Design review of the part built by this model. Coordinates are the model's own, in mm. Round coordinates to 2 decimals unless told otherwise and drop trailing zeros. Loops run counter-clockwise (first coordinate to the right, second up) from the corner with the lowest first, then second, coordinate; pieces in that order, holes last. Notation, with made-up numbers: (84, 86.5) -> (121, 86.5) arc R13 cw to (121, 106.5) -> close; hole circle Ø9 at (82, -27). An arc over 180 degrees is marked (long way). Write each question's results on one line, items separated by ' | '. Start each with the question number.
from build123d import *

# Parameters (mm, degrees)
SKETCH1_W                  = 187
SKETCH1_H                  = 137
BOSS_EXTRUDE1_DEPTH        = 4.87
F_7_0_7_DIAMETER_HOLE1_D   = 7
F_3_2_3_2_DIAMETER_HOLE1_D = 3.2
SKETCH6_W                  = 58
SKETCH6_H                  = 101.3
BOSS_EXTRUDE2_DEPTH        = 1
SKETCH7_W                  = 12.3
SKETCH7_H                  = 11
BOSS_EXTRUDE3_DEPTH        = 1
SKETCH8_W                  = 203.41830683
SKETCH8_H                  = 2.7
CUT_EXTRUDE1_DEPTH         = 1
FILLET1_R                  = 7


with BuildPart() as part:
    # Sketch1 → Boss-Extrude1 (new body)
    with BuildSketch(Plane.XY):
        Rectangle(SKETCH1_W, SKETCH1_H)
    extrude(amount=BOSS_EXTRUDE1_DEPTH)

    # Ø7.0 (7) Diameter Hole1 (through all)
    with Locations(Plane.XY.offset(4.87)):
        with Locations((-28.5, 62), (-85.5, 62), (28.5, 62), (85.5, 62), (85.5, -62), (28.5, -62), (-85.5, -62), (-28.5, -62)):
            Hole(F_7_0_7_DIAMETER_HOLE1_D / 2)

    # Ø3.2 (3.2) Diameter Hole1 (through all)
    with Locations(Plane.XY.offset(4.87)):
        with Locations((-57.1, 61.02), (57.1, 60.975), (57.1, -60.975), (-57.1, -61.02)):
            Hole(F_3_2_3_2_DIAMETER_HOLE1_D / 2)

    # Sketch6 → Boss-Extrude2 (add)
    with BuildSketch(Plane.XY.offset(4.87)):
        with Locations((-61, 0)):
            Rectangle(SKETCH6_W, SKETCH6_H)
        Rectangle(SKETCH6_W, SKETCH6_H)
        with Locations((61, 0)):
            Rectangle(SKETCH6_W, SKETCH6_H)
    extrude(amount=BOSS_EXTRUDE2_DEPTH)

    # Sketch7 → Boss-Extrude3 (add)
    with BuildSketch(Plane.XY.offset(4.87)):
        with Locations((-68.55, -57.85)):
            Rectangle(SKETCH7_W, SKETCH7_H)
        with Locations((-45.24, -57.85)):
            Rectangle(SKETCH7_W, SKETCH7_H)
        with Locations((-11.54, -57.85)):
            Rectangle(SKETCH7_W, SKETCH7_H)
    extrude(amount=BOSS_EXTRUDE3_DEPTH)

    # Sketch8 → Cut-Extrude1 (cut)
    with BuildSketch(Plane.XY.offset(5.87)):
        Rectangle(SKETCH8_W, SKETCH8_H)
    extrude(amount=-CUT_EXTRUDE1_DEPTH, mode=Mode.SUBTRACT)

    # Fillet1
    fillet1_edges = [part.edges().sort_by_distance(p)[0] for p in [
        (93.5, -68.5, 2.435),
        (-93.5, -68.5, 2.435),
        (-93.5, 68.5, 2.435),
        (93.5, 68.5, 2.435),
    ]]
    fillet(fillet1_edges, radius=FILLET1_R)


solid = part.part
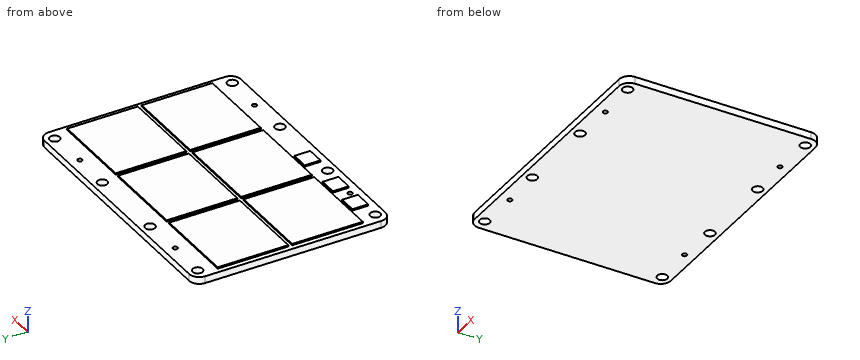
1) To check wall thickness, follow line 1 (Y direction, x = -85.5, z = 1.2); line 2 (X direction, y = 4, z = 5.35); line 3 (Y direction, x = 57.1, z = 1.9) (3 decimals). State the ranges of each line that lie inside material, in increasing order. Write a range as from..to.
2) Insertion check: pin 1 (0.8 mm diameter, centred on x = 58, z = 5.5, fed in from +Y); pin 2 (4 mm diameter, centred on x = 28.5, y = 62, fed in from +Z); pin 3 (1.1 mm diameter, centred on y = -37.5, z = 5.5, fed in from -X); pin 4 (0.8 mm diameter, centred on y = 15, z = 5.5, fed in from +X). Each pin has a flat end and moves straight along its axis. Give the tip position at first contact, or say it passes through.
3) Take a section at A-A (x = -12). Write out the cut boundary in (y, z), plus the area to 3 significant figures.
Geometry check:
1) line 1: y = -68.5..-65.5, -58.5..58.5, 65.5..68.5 | line 2: x = -90..-32, -29..29, 32..90 | line 3: y = -68.5..-62.575, -59.375..59.375, 62.575..68.5
2) pin 1: stops at y = 50.65 | pin 2: passes through | pin 3: stops at x = -90 | pin 4: stops at x = 90
3) outline: (-68.5, 0) -> (68.5, 0) -> (68.5, 4.87) -> (50.65, 4.87) -> (50.65, 5.87) -> (1.35, 5.87) -> (1.35, 4.87) -> (-1.35, 4.87) -> (-1.35, 5.87) -> (-50.65, 5.87) -> (-50.65, 4.87) -> (-52.35, 4.87) -> (-52.35, 5.87) -> (-63.35, 5.87) -> (-63.35, 4.87) -> (-68.5, 4.87) -> close | area: 777 mm^2
